from build123d import *

# Parameters (mm, degrees)
LOWER_ARMS_25MM_DEPTH                 = 25
HUB_BOSS_SKETCH_32_R                  = 32
HUB_BOSS_32_DEPTH                     = 31
UPPER_START                           = -20
UPPER_ARMS_20MM_DEPTH                 = 20
HUB_COLLAR_SKETCH_32_R                = 32
HUB_COLLAR_32X4_DEPTH                 = 4
KEYED_HUB_BORE_DEPTH                  = 70
UPPER_ARM_PADS_SKETCH_3X_13_R         = 13
UPPER_ARM_PADS_3X_13_DEPTH            = 4
UPPER_ARM_HOLES_SKETCH_3X_8_R         = 8
UPPER_ARM_HOLES_3X_8_DEPTH            = 30
LOWER_ARM_COUNTERBORES_SKETCH_2X_12_R = 12
LOWER_ARM_COUNTERBORES_2X_12_DEPTH    = 6
LOWER_ARM_HOLES_SKETCH_2X_7_R         = 7
LOWER_ARM_HOLES_2X_7_DEPTH            = 20


with BuildPart() as part:
    # Lower Arms Profile → Lower Arms 25mm (new body)
    with BuildSketch(Plane.XY):
        with BuildLine():
            Line((-57.296551724, -34.95862069), (-27.674482759, 16.066206897))
            ThreePointArc((-27.674482759, 16.066206897), (0, 32), (27.674482759, 16.066206897))
            Line((27.674482759, 16.066206897), (57.296551724, -34.95862069))
            ThreePointArc((57.296551724, -34.95862069), (57.332449137, -54.979288897), (40, -65))
            Line((40, -65), (-40, -65))
            ThreePointArc((-40, -65), (-57.332449137, -54.979288897), (-57.296551724, -34.95862069))
        make_face()
    extrude(amount=LOWER_ARMS_25MM_DEPTH)

    # Hub Boss Sketch Ø32 → Hub Boss Ø32 (add)
    with BuildSketch(Plane.XY.offset(25)):
        with Locations(Location((0, 0, 0), (0, 0, 149.863023681))):
            Circle(HUB_BOSS_SKETCH_32_R)
    extrude(amount=HUB_BOSS_32_DEPTH)

    # Upper Arms Profile → Upper Arms 20mm (add)
    with BuildSketch(Plane.XY.offset(56).offset(UPPER_START)):
        with BuildLine():
            Line((-20, -24.979991994), (-20, -75))
            ThreePointArc((-20, -75), (0, -95), (20, -75))
            Line((20, -75), (20, -24.979991994))
            ThreePointArc((20, -24.979991994), (0, -32), (-20, -24.979991994))
        make_face()
        with BuildLine():
            ThreePointArc((-54.951905284, 54.820508076), (-82.27241336, 47.5), (-74.951905284, 20.179491924))
            Line((-74.951905284, 20.179491924), (-31.633307653, -4.830512079))
            ThreePointArc((-31.633307653, -4.830512079), (-27.712812921, 16), (-11.633307653, 29.810504072))
            Line((-11.633307653, 29.810504072), (-54.951905284, 54.820508076))
        make_face()
        with BuildLine():
            ThreePointArc((75.864190859, 20.73927139), (81.712633894, 48.412285575), (54.039619709, 54.26072861))
            Line((54.039619709, 54.26072861), (14.507199018, 28.522643227))
            ThreePointArc((14.507199018, 28.522643227), (29.291756215, 12.883827763), (30.827638328, -8.582349045))
            Line((30.827638328, -8.582349045), (75.864190859, 20.73927139))
        make_face()
    extrude(amount=UPPER_ARMS_20MM_DEPTH)

    # Hub Collar Sketch Ø32 → Hub Collar Ø32x4 (add)
    with BuildSketch(Plane.XY.offset(56)):
        with Locations(Location((0, 0, 0), (0, 0, 149.863023681))):
            Circle(HUB_COLLAR_SKETCH_32_R)
    extrude(amount=HUB_COLLAR_32X4_DEPTH)

    # Keyed Bore Sketch → Keyed Hub Bore (cut)
    with BuildSketch(Plane.XY.offset(60)):
        with BuildLine():
            Line((-2.5, -24), (2.5, -24))
            Line((2.5, -24), (2.5, -19.843134833))
            ThreePointArc((2.5, -19.843134833), (0, 20), (-2.5, -19.843134833))
            Line((-2.5, -19.843134833), (-2.5, -24))
        make_face()
    extrude(amount=-KEYED_HUB_BORE_DEPTH, mode=Mode.SUBTRACT)

    # Upper Arm Pads Sketch 3xØ13 → Upper Arm Pads 3xØ13 (add)
    with BuildSketch(Plane.XY.offset(56)):
        with Locations((-64.951905284, 37.5)):
            Circle(UPPER_ARM_PADS_SKETCH_3X_13_R)
        with Locations((64.951905284, 37.5)):
            Circle(UPPER_ARM_PADS_SKETCH_3X_13_R)
        with Locations((0, -75)):
            Circle(UPPER_ARM_PADS_SKETCH_3X_13_R)
    extrude(amount=UPPER_ARM_PADS_3X_13_DEPTH)

    # Upper Arm Holes Sketch 3xØ8 → Upper Arm Holes 3xØ8 (cut)
    with BuildSketch(Plane.XY.offset(60)):
        with Locations((-64.951905284, 37.5)):
            Circle(UPPER_ARM_HOLES_SKETCH_3X_8_R)
        with Locations((64.951905284, 37.5)):
            Circle(UPPER_ARM_HOLES_SKETCH_3X_8_R)
        with Locations((0, -75)):
            Circle(UPPER_ARM_HOLES_SKETCH_3X_8_R)
    extrude(amount=-UPPER_ARM_HOLES_3X_8_DEPTH, mode=Mode.SUBTRACT)

    # Lower Arm Counterbores Sketch 2xØ12 → Lower Arm Counterbores 2xØ12 (cut)
    with BuildSketch(Plane.XY.offset(25)):
        with Locations((-40, -45)):
            Circle(LOWER_ARM_COUNTERBORES_SKETCH_2X_12_R)
        with Locations((40, -45)):
            Circle(LOWER_ARM_COUNTERBORES_SKETCH_2X_12_R)
    extrude(amount=-LOWER_ARM_COUNTERBORES_2X_12_DEPTH, mode=Mode.SUBTRACT)

    # Lower Arm Holes Sketch 2xØ7 → Lower Arm Holes 2xØ7 (cut)
    with BuildSketch(Plane.XY.offset(19)):
        with Locations((-40, -45)):
            Circle(LOWER_ARM_HOLES_SKETCH_2X_7_R)
        with Locations((40, -45)):
            Circle(LOWER_ARM_HOLES_SKETCH_2X_7_R)
    extrude(amount=-LOWER_ARM_HOLES_2X_7_DEPTH, mode=Mode.SUBTRACT)


solid = part.part
Here's how the part is built. I have some questions about the finished solid (model axes, mm). A direction names the side the tool comes from. Round coordinates to 2 decimals unless told otherwise and drop trailing zeros. Loops run counter-clockwise (first coordinate to the right, second up) from the corner with the lowest first, then second, coordinate; pieces in that order, holes last.
1. If I drill on line 1 along Y through (x, z) = (0, 47); line 2 along Z through (x, y) = (-34, 0.5); line 3 along Z through (x, y) = (-46.5, 15), over which ranges is the centre line in solid material (lowest first)?
Answer list:
line 1: y = -95 to -83, -67 to -24, 20 to 32
line 2: z = 0 to 25, 36 to 56
line 3: z = 36 to 56
2. For P1, Ø20, axis at x = -17.5, z = 14, coming from the -Y side; P2, Ø3, axis at x = 67.5, z = 35.5, coming from the -Y side; P3, Ø16, axis at x = -40, y = -45, coming from the +Z side; P4, Ø10, axis at y = 37, z = 34, coming from the +X side, each with a flat end and sliding along its axis, tell me the tip position at first contact or that it passes through.
Answer list:
P1: stops at y = -65
P2: stops at y = 14.37
P3: stops at z = 19
P4: stops at x = 84.95
3. If we section it at B-B on x = 0: Write out the boundary of the cut face in (y, z), plus the area to 4 significant figures.
Answer list:
outline: (-95, 36) - (-83, 36) - (-83, 60) - (-88, 60) - (-88, 56) - (-95, 56) - close; (-67, 36) - (-32, 36) - (-32, 25) - (-65, 25) - (-65, 0) - (-24, 0) - (-24, 60) - (-32, 60) - (-32, 56) - (-62, 56) - (-62, 60) - (-67, 60) - close; (20, 0) - (32, 0) - (32, 60) - (20, 60) - close
area: 3,005 mm2
4. If we section it at C-C on y = 37.5: Write out the boundary of the cut face in (x, z).
Answer list:
outline: (-84.95, 36) - (-72.95, 36) - (-72.95, 60) - (-77.95, 60) - (-77.95, 56) - (-84.95, 56) - close; (-56.95, 36) - (-24.95, 36) - (-24.95, 56) - (-51.95, 56) - (-51.95, 60) - (-56.95, 60) - close; (28.3, 36) - (56.95, 36) - (56.95, 60) - (51.95, 60) - (51.95, 56) - (28.3, 56) - close; (72.95, 36) - (84.95, 36) - (84.95, 56) - (77.95, 56) - (77.95, 60) - (72.95, 60) - close
5. Which directions (+Z, -Z, +X, -X, +Y, -Y) give clear straight access to the entire face, cutting with the end or side of a thin tool? Please do faces 1 (the face through (-1.69, -62.11, 57.97)), 2 (the face through (-42.69, -9.8, 12.32)), 3 (the face through (1, -65, 12)), 4 (the face through (2.5, -22, 30)).
Answer list:
face 1: +Z
face 2: -Z, -X, +Y
face 3: -Z, +X, -X, -Y
face 4: +Z, -Z
6. We'd pull the mould along Z, two halves only. Please class faces 5 (the face through (-49, 27, 56)), 6 (the face through (0, -59, 36)), 7 (the face through (-2.5, -22, 30)): +Z half, -Z half, draft (parallel to the pull), parting line (faces both ways), or undercut.
Answer list:
face 5: +Z half
face 6: undercut
face 7: draft
7. If we section it at D-D on y = -81: Write out the boundary of the cut face in (x, z), plus the area to 3 significant figures.
Answer list:
outline: (-19.08, 36) - (-5.29, 36) - (-5.29, 60) - (-11.53, 60) - (-11.53, 56) - (-19.08, 56) - close; (5.29, 36) - (19.08, 36) - (19.08, 56) - (11.53, 56) - (11.53, 60) - (5.29, 60) - close
area: 601 mm2
8. If we section it at A-A on z = 10: Write out the boundary of the cut face in (x, y), plus the area to 3 significant figures.
Answer list:
outline: (-57.3, -34.96) arc R20 ccw to (-40, -65) - (40, -65) arc R20 ccw to (57.3, -34.96) - (27.67, 16.07) arc R32 ccw to (-27.67, 16.07) - close; hole circle Ø14 at (-40, -45); hole (-2.5, -24) - (2.5, -24) - (2.5, -19.84) arc R20 ccw (long way) to (-2.5, -19.84) - close; hole circle Ø14 at (40, -45)
area: 6,790 mm2
